Read the model definition and answer for the solid it produces. Units are mm, in the model's axes. Face numbers are marked on the shaded views. A direction names the side the tool comes from. Give positions to 0.01 mm unless a question says otherwise; leave off trailing zeros. Order: outer loops, then holes, each group sorted by start corner. A loop starts at its lowest first (then second) coordinate and runs counter-clockwise, first axis right, second up. Notation, with made-up numbers: M 40,-2 L 92,-2 A14 cw 92,6 Z; hole C 79.25,89 d5. An arc over 180 degrees is marked long. Write item = value, one per line. Start each with the question number.
from build123d import *

# Parameters (mm, degrees)
BASE_PLATE_SKETCH_W        = 140
BASE_PLATE_SKETCH_H        = 90
BASE_PLATE_DEPTH           = 40
GLAND_BOSS_SKETCH_R        = 30
GLAND_BOSS_SKETCH_R_2      = 20
GLAND_BOSS_DEPTH           = 60
FORK_START                 = -30
FORK_CUTOUT_DEPTH          = 30
BORE_AND_HOLE_CUT_REACH    = 94.331
BORE_AND_HOLE_CUT_SKETCH_R = 8
BORE_AND_HOLE_CUT_SKETCH_W = 20
BORE_AND_HOLE_CUT_SKETCH_H = 40
SUPPORT_WEB_SKETCH_W       = 15.952624903
SUPPORT_WEB_SKETCH_H       = 15
SUPPORT_WEB_DEPTH          = 50
LIP_SKETCH_R               = 20
LIP_SKETCH_R_2             = 8
LIP_10MM_DEPTH             = 10


with BuildPart() as part:
    # Base Plate Sketch → Base Plate (new body)
    with BuildSketch(Plane(origin=(0, 0, 0), x_dir=(1, 0, 0), z_dir=(0, 1, 0))):
        Rectangle(BASE_PLATE_SKETCH_W, BASE_PLATE_SKETCH_H)
    extrude(amount=BASE_PLATE_DEPTH)

    # Gland Boss Sketch → Gland Boss (add)
    with BuildSketch(Plane(origin=(0, 0, 0), x_dir=(1, 0, 0), z_dir=(0, 1, 0))):
        with Locations(Location((0, 0, 0), (0, 0, 90))):
            Circle(GLAND_BOSS_SKETCH_R)
        with Locations(Location((0, 0, 0), (0, 0, 90))):
            Circle(GLAND_BOSS_SKETCH_R_2, mode=Mode.SUBTRACT)
    extrude(amount=GLAND_BOSS_DEPTH)

    # Fork Cutout Sketch → Fork Cutout (cut)
    with BuildSketch(Plane(origin=(0, 40, 0), x_dir=(1, 0, 0), z_dir=(0, 1, 0)).offset(FORK_START)):
        with BuildLine():
            Line((-70, 20), (-60, 20))
            Line((-60, 20), (-60, 35))
            Line((-60, 35), (-30, 35))
            Line((-30, 35), (-30, 45))
            Line((-30, 45), (30, 45))
            Line((30, 45), (-11.538461538, 27.692307692))
            ThreePointArc((-11.538461538, 27.692307692), (-30, 0), (-11.538461538, -27.692307692))
            Line((-11.538461538, -27.692307692), (30, -45))
            Line((30, -45), (-30, -45))
            Line((-30, -45), (-30, -35))
            Line((-30, -35), (-60, -35))
            Line((-60, -35), (-60, -20))
            Line((-60, -20), (-70, -20))
            Line((-70, -20), (-70, 20))
        make_face()
    extrude(amount=FORK_CUTOUT_DEPTH, mode=Mode.SUBTRACT)

    # Bore and Hole Cut Sketch → Bore and Hole Cut (cut, up to next)
    with BuildSketch(Plane(origin=(0, 40, 0), x_dir=(1, 0, 0), z_dir=(0, 1, 0)), mode=Mode.PRIVATE) as bore_and_hole_cut_sk1:
        with Locations(Location((0, 0, 0), (0, 0, 270))):
            Circle(BORE_AND_HOLE_CUT_SKETCH_R)
    bore_and_hole_cut_tool1 = extrude(bore_and_hole_cut_sk1.sketch, amount=-BORE_AND_HOLE_CUT_REACH, mode=Mode.PRIVATE) & part.part
    # Bore and Hole Cut Sketch → Bore and Hole Cut (cut, up to next)
    with BuildSketch(Plane(origin=(0, 40, 0), x_dir=(1, 0, 0), z_dir=(0, 1, 0)), mode=Mode.PRIVATE) as bore_and_hole_cut_sk2:
        with Locations(Location((50, 0, 0), (0, 0, 270))):
            Circle(BORE_AND_HOLE_CUT_SKETCH_R)
    bore_and_hole_cut_tool2 = extrude(bore_and_hole_cut_sk2.sketch, amount=-BORE_AND_HOLE_CUT_REACH, mode=Mode.PRIVATE) & part.part
    # Bore and Hole Cut Sketch → Bore and Hole Cut (cut, up to next)
    with BuildSketch(Plane(origin=(0, 40, 0), x_dir=(1, 0, 0), z_dir=(0, 1, 0)), mode=Mode.PRIVATE) as bore_and_hole_cut_sk3:
        with Locations((-60, 0)):
            Rectangle(BORE_AND_HOLE_CUT_SKETCH_W, BORE_AND_HOLE_CUT_SKETCH_H)
    bore_and_hole_cut_tool3 = extrude(bore_and_hole_cut_sk3.sketch, amount=-BORE_AND_HOLE_CUT_REACH, mode=Mode.PRIVATE) & part.part
    add(bore_and_hole_cut_tool1.solids().sort_by_distance((0, 40, 0))[0], mode=Mode.SUBTRACT)
    add(bore_and_hole_cut_tool2.solids().sort_by_distance((50, 40, 0))[0], mode=Mode.SUBTRACT)
    add(bore_and_hole_cut_tool3.solids().sort_by_distance((-60, 40, 0))[0], mode=Mode.SUBTRACT)

    # Support Web Sketch → Support Web (add)
    with BuildSketch(Plane(origin=(0, 60, 0), x_dir=(1, 0, 0), z_dir=(0, 1, 0))):
        with Locations((-37.023687548, 0)):
            Rectangle(SUPPORT_WEB_SKETCH_W, SUPPORT_WEB_SKETCH_H)
    extrude(amount=-SUPPORT_WEB_DEPTH)

    # Tapered Cut Start Profil for Tapered Lof → Tapered Lofted Cut section 0
    with BuildSketch(Plane(origin=(0, 60, 0), x_dir=(1, 0, 0), z_dir=(0, 1, 0))):
        with BuildLine():
            Line((-29.047375097, 7.5), (-45, 7.5))
            Line((-45, 7.5), (-45, -7.5))
            Line((-45, -7.5), (-29.047375097, -7.5))
            # circular arc as an exact rational Bezier (weights 1, cos(half-angle), 1)
            Bezier((-29.047375097, -7.5), (-30.98386677, 0), (-29.047375097, 7.5), weights=[1, 0.968245837, 1])
        make_face()
    # Tapered Cut End Profile → Tapered Lofted Cut section 1
    with BuildSketch(Plane(origin=(0, 10, 0), x_dir=(1, 0, 0), z_dir=(0, 1, 0))):
        with BuildLine():
            Line((-50, 15.482090991), (-45, 15.482090991))
            Line((-45, 15.482090991), (-45, -14.57582225))
            Line((-45, -14.57582225), (-50, -14.57582225))
            Line((-50, -14.57582225), (-50, 15.482090991))
        make_face()
    loft(mode=Mode.SUBTRACT)

    # Lip Sketch → Lip 10mm (add)
    with BuildSketch(Plane(origin=(0, 40, 0), x_dir=(1, 0, 0), z_dir=(0, 1, 0))):
        with Locations(Location((0, 0, 0), (0, 0, 270))):
            Circle(LIP_SKETCH_R)
        with Locations(Location((0, 0, 0), (0, 0, 270))):
            Circle(LIP_SKETCH_R_2, mode=Mode.SUBTRACT)
    extrude(amount=LIP_10MM_DEPTH)


solid = part.part
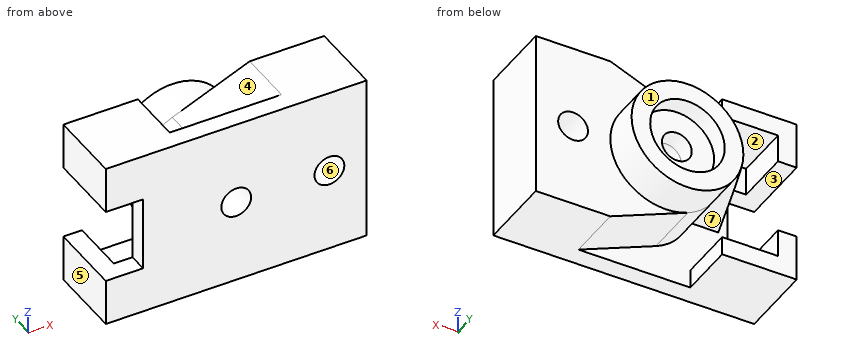
1) For a pull along X with two mould halves and no side action, classify the marked faces 4, 5, 6 and 7 as pulls with the +X half, pulls with the -X half, needs draft (parallel to the pull), parting line crosses it, or undercut.
2) Each of these flat-tipped pins is pushed along its axis until it touches: P1, Ø1, axis at x = -10.5, y = 51.5, coming from the +Z side; P2, Ø4, axis at x = 25, y = 30.5, coming from the -Z side; P3, Ø12, axis at x = -5, z = -9.5, coming from the +Y side; P4, Ø9.5, axis at x = 50, z = 0, coming from the -Y side. Where does it stop, or does it pass through?
3) Find section C-C on y = 35. Count the separate pieces of the cut face and the enclosed holes in it, plus the area to 3 significant figures.
4) For the marked faces 1, 2 and 3, determine the directions among +Z, -Z, +X, -X, +Y, -Y from which every point of the face is accessible in a straight line to the end or side of a thin tool.
5) Find section A-A on x = 0. Determine the outline of the cut face in (y, z).
6) Find section D-D on x = 50. Determine the outline of the cut face in (y, z), plus the area to 3 significant figures.
7) Find section B-B on z = -33. Determine the outline of the cut face in (x, y).
8) Find the intervals of material crossed by probe 1 along X at (y, z) = (8.5, -0.5); probe 2 along Z at (x, y) = (0, 56); probe 3 along X at (y, z) = (11, 0), in increasing order. Write a range as [from, to].
Numbers:
q1.face_4 = undercut
q1.face_5 = pulls with the -X half
q1.face_6 = undercut
q1.face_7 = needs draft
q2.P1 = 28.28
q2.P2 = -43.75
q2.P3 = 50
q2.P4 = through
q3.separate_pieces = 3
q3.enclosed_holes = 2
q3.area = 8,170 mm2
q4.face_1 = +Z, -Z, +X, -X, +Y
q4.face_2 = +Y
q4.face_3 = -X, +Y, -Y
q5.outline = M 0,-45 L 10,-45 L 10,-32.5 L 40,-32.5 L 40,-30 L 60,-30 L 60,-20 L 50,-20 L 50,-8 L 0,-8 Z; M 0,8 L 50,8 L 50,20 L 60,20 L 60,30 L 40,30 L 40,32.5 L 10,32.5 L 10,45 L 0,45 Z
q6.outline = M 0,-45 L 40,-45 L 40,-8 L 0,-8 Z; M 0,8 L 40,8 L 40,45 L 0,45 Z
q6.area = 2,960 mm2
q7.outline = M -70,0 L 70,0 L 70,40 L 1.2,40 L 1.2,10 L -60,10 L -60,40 L -70,40 Z
q8.probe_1 = [-50, -7.98], [7.98, 42.02], [57.98, 70]
q8.probe_2 = [-30, -20], [20, 30]
q8.probe_3 = [-44.7, -8], [8, 42], [58, 70]
